The model under review builds one solid part; all positions refer to its coordinate system, in mm. A direction names the side the tool comes from. Round coordinates to 2 decimals unless told otherwise and drop trailing zeros. Order: outer loops, then holes, each group sorted by start corner. A loop starts at its lowest first (then second) coordinate and runs counter-clockwise, first axis right, second up.
```python
from build123d import *

# Parameters (mm, degrees)
SKETCH1_R             = 25
SKETCH1_R_2           = 20
BOSS_EXTRUDE1_DEPTH   = 10
BOSS_EXTRUDE1_2_DEPTH = 10
BOSS_EXTRUDE1_3_DEPTH = 10
BOSS_EXTRUDE2_DEPTH   = 10


with BuildPart() as part:
    # Sketch1 → Boss-Extrude1 (new body)
    with BuildSketch(Plane.XY):
        with Locations((-659.884196758, -20)):
            Circle(SKETCH1_R)
        with Locations((-659.884196758, -20)):
            Circle(SKETCH1_R_2, mode=Mode.SUBTRACT)
    extrude(amount=-BOSS_EXTRUDE1_DEPTH)



with BuildPart() as body_2:
    # Sketch1 → Boss-Extrude1 2 (new body)
    with BuildSketch(Plane.XY):
        with Locations((-539.884196758, -20)):
            Circle(SKETCH1_R)
        with Locations((-539.884196758, -20)):
            Circle(SKETCH1_R_2, mode=Mode.SUBTRACT)
    extrude(amount=-BOSS_EXTRUDE1_2_DEPTH)


with BuildPart() as body_3:
    # Sketch1 → Boss-Extrude1 3 (new body)
    with BuildSketch(Plane.XY):
        with Locations((-539.884196758, -160)):
            Circle(SKETCH1_R)
        with Locations((-539.884196758, -160)):
            Circle(SKETCH1_R_2, mode=Mode.SUBTRACT)
    extrude(amount=-BOSS_EXTRUDE1_3_DEPTH)


with BuildPart() as part_1:
    add(part.part)

    add(body_2.part)  # Boss-Extrude2 merges body 2

    add(body_3.part)  # Boss-Extrude2 merges body 3
    # Sketch2 → Boss-Extrude2 (add)
    with BuildSketch(Plane.XY):
        Polygon((-544.884196758, -222.781745931), (-467.102450828, -145), (-467.102450828, -35), (-544.884196758, 42.781745931), (-654.884196758, 42.781745931), (-732.665942689, -35), (-732.665942689, -145), (-654.884196758, -222.781745931), align=None)
    extrude(amount=BOSS_EXTRUDE2_DEPTH)


solid = part_1.part
```
(1) Insertion check: pin 1 (10 mm diameter, centred on x = -664, z = 0, fed in from -Y); pin 2 (4 mm diameter, centred on y = -7.5, z = -7.5, fed in from -X); pin 3 (12 mm diameter, centred on x = -670, y = -19.5, fed in from -Z). Each pin has a flat end and moves straight along its axis. Give the tip position at first contact, or say it passes through.
Data:
pin 1: stops at y = -218.67
pin 2: stops at x = -682.57
pin 3: stops at z = 0
(2) To check wall thickness, follow probe 1 along Z at (x, y) = (-542, -103); probe 2 along Y at (x, z) = (-670, -6.5); probe 3 along X at (y, z) = (-149, -1). State the ranges of each line that lie inside material, in increasing order.
Data:
probe 1: z = 0 to 10
probe 2: y = -42.86 to -37.25, -2.75 to 2.86
probe 3: x = -562.33 to -556.59, -523.18 to -517.43
(3) Draft analysis for pull direction Y (two halves, no side actions). For faces 1 (the cylindrical face through (-636.04, -12.49, -4.93)), 2 (the cylindrical face through (-559.865, -19.121, -4.93)), 3 (the cylindrical face through (-559.865, -159.121, -4.93)), 4 (the flat face through (-693.231, 4.435, 4.93)), state which applies: pulls with the +Y half, pulls with the -Y half, needs draft (parallel to the pull), parting line crosses it, or undercut.
Data:
face 1: parting line crosses it
face 2: undercut
face 3: undercut
face 4: pulls with the +Y half
(4) Consider section D-D (y = -123.5). Write out the cut boundary in (x, z).
Data:
outline: (-732.67, 0) - (-467.1, 0) - (-467.1, 10) - (-732.67, 10) - close
(5) Consider section A-A (z = 4.25). Write out the cut boundary in (x, y).
Data:
outline: (-732.67, -145) - (-654.88, -222.78) - (-544.88, -222.78) - (-467.1, -145) - (-467.1, -35) - (-544.88, 42.78) - (-654.88, 42.78) - (-732.67, -35) - close
(6) For faces 5 (the flat face through (-540, -20, 0)), 6 (the flat face through (-467.102, -91, 5)), list the 3-axis set-ups (+Z, -Z, +X, -X, +Y, -Y) from which the entire face can be reached by the end or side of a thin tool; tool diameter is ignored.
Data:
face 5: -Z
face 6: +Z, -Z, +X, +Y, -Y
(7) Consider section B-B (y = -160). Write out the cut boundary in (x, z).
Data:
outline: (-717.67, 0) - (-564.88, 0) - (-564.88, -10) - (-559.88, -10) - (-559.88, 0) - (-519.88, 0) - (-519.88, -10) - (-514.88, -10) - (-514.88, 0) - (-482.1, 0) - (-482.1, 10) - (-717.67, 10) - close
(8) Consider section C-C (x = -615.5). Write out the cut boundary in (y, z).
Data:
outline: (-222.78, 0) - (42.78, 0) - (42.78, 10) - (-222.78, 10) - close
